Verification items for the finished model (mm, model axes). A direction names the side the tool comes from. Coordinates: 2 decimals unless noted, no trailing zeros. Loops run counter-clockwise (first coordinate to the right, second up) from the corner with the lowest first, then second, coordinate; pieces in that order, holes last.
Q1. Sectioned sample at A-A (z = 17). Enter the section's corners in (x, y), then the cut area to 3 significant figures.
Q2. Mould release check, pull along Z, two halves, no side actions. Record for faces 1 (the face through (-3, 5.78, 27.29)), 2 (the face through (0, 0, 0)), 3 (the face through (-5.328, -1.678, 84.516)): +Z half, -Z half, draft (parallel to the pull), parting line (faces both ways), or undercut.
Q3. Material ranges on probe 1 along Z at (x, y) = (5.5, -10.75); probe 2 along X at (y, z) = (-0.25, 113); probe 3 along X at (y, z) = (-3.75, 130.5), recorded low to high.
Q4. Go/stop test with flat-tipped pins: P1, Ø8, axis at x = 7, z = 38.5, coming from the +Y side; P2, Ø5, axis at x = 2, z = 85.5, coming from the +Y side; P3, Ø6, axis at y = -11, z = 72.5, coming from the +X side; P4, Ø1.5, axis at y = 3, z = 126.5, coming from the -X side. Record where each tip stops, or that it passes through.
Q5. Sectioned sample at B-B (z = 66). Enter the section's corners in (x, y).
Q6. Access from +Z, -Z, +X, -X, +Y, -Y to the whole of each face (thin tool, end or side, straight path). Record for faces 4 (the face through (6.633, -6.083, 15.07)), 5 (the face through (-14.985, 0.66, 4.93)).
```python
from build123d import *

# Parameters (mm, degrees)
SKETCH1_R           = 15
BOSS_EXTRUDE1_DEPTH = 10


with BuildPart() as part:
    # Sketch1 → Boss-Extrude1 (new body)
    with BuildSketch(Plane.XY):
        Circle(SKETCH1_R)
    extrude(amount=BOSS_EXTRUDE1_DEPTH)

    # Sketch2 → Revolve1 (revolve)
    with BuildSketch(Plane(origin=(0, 0, 0), x_dir=(1, 0, 0), z_dir=(0, 1, 0)), mode=Mode.PRIVATE) as revolve1_sk:
        Polygon((9, -10), (9, -20), (5.585921345, -30), (5.585921345, -137.526835229), (0, -150), (0, -10), align=None)
    revolve(revolve1_sk.sketch.rotate(Axis((0, 0, -14.229599779), (0, 0, 1)), 180), axis=Axis((0, 0, -14.229599779), (0, 0, 1)))


solid = part.part
```
Geometry check:
1. outline: circle Ø18 at (0, 0)
1. area: 254 mm2
2. face 1: +Z half
2. face 2: -Z half
2. face 3: draft
3. probe 1: z = 0 to 10
3. probe 2: x = -5.58 to 5.58
3. probe 3: x = -4.14 to 4.14
4. P1: stops at y = 4.71
4. P2: stops at y = 5.59
4. P3: passes through
4. P4: stops at x = -5.11
5. outline: circle Ø11.17 at (0, 0)
6. face 4: +Z
6. face 5: +Z, -Z
